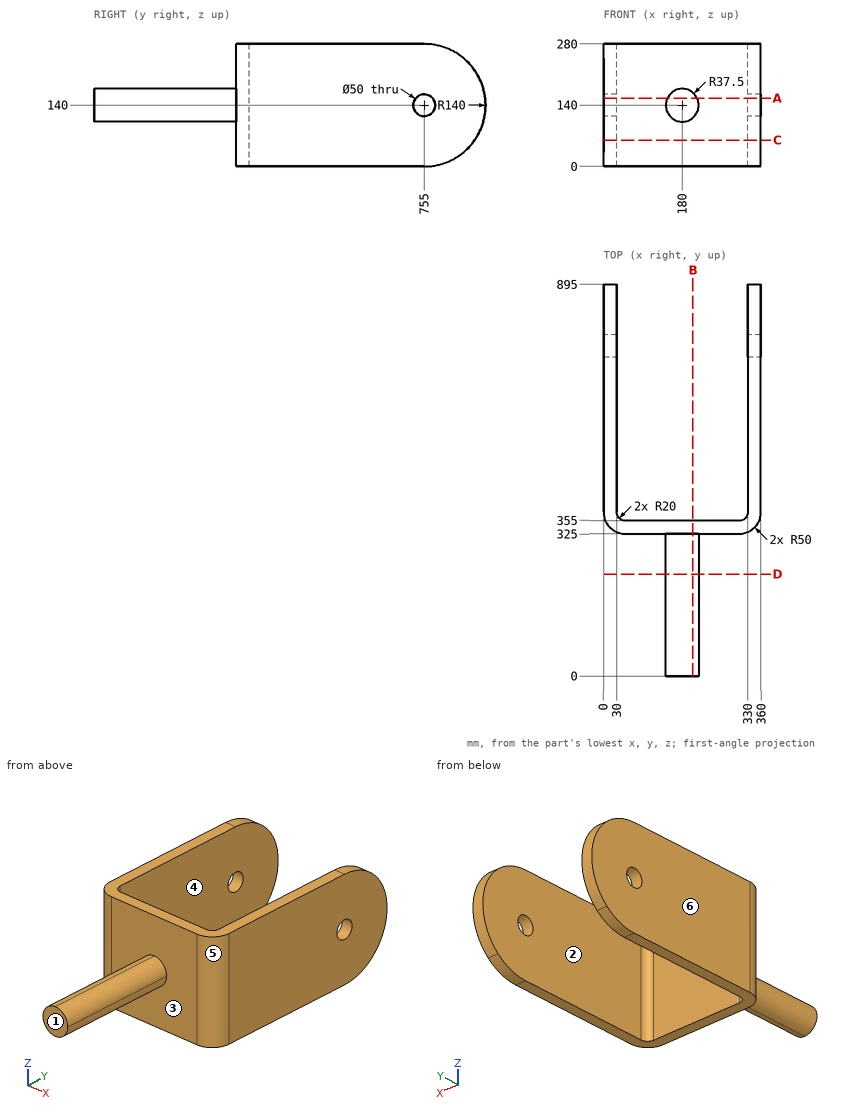
Can you work these out from the drawing? Everything is in mm from the part's minimum corner. A direction names the side the tool comes from. Round coordinates to 2 decimals unless told otherwise and drop trailing zeros. Loops run counter-clockwise (first coordinate to the right, second up) from the corner with the lowest first, then second, coordinate; pieces in that order, holes last. Notation, with made-up numbers: (1.25, -22.75) - (27.25, -22.75) arc R10 cw to (27.25, -18.75) - close; hole circle Ø2 at (18, 40.5). An arc over 180 degrees is marked (long way). Answer in a Markdown table with one row per item. Add a question column.
(1) If we section it at C-C (z = 60): Please give me the cut outline in (x, y), plus the area to 3 significant figures.
(2) If we mould it in two halves opening along X, with no side actions, what happens to the marked faces 4, 5 and 6? For each: pulls with the +X half, pulls with the -X half, needs draft (parallel to the pull), parting line crosses it, or undercut.
(3) I need wall thicknesses on line 1 along X through (y, z) = (641, 182.5); line 2 along Z through (x, y) = (17, 755); line 3 along Y through (x, z) = (135.5, 106.5). Which ranges of each line are inside material? Lowest first, please.
(4) If we section it at A-A (z = 156): Please give me the cut outline in (x, y).
(5) For the marked faces 1, 2 and 3, which set-ups out of +Z, -Z, +X, -X, +Y, -Y let a thin tool reach every point of the face, with its end or its side?
(6) I'm going to push flat-ended pins straight in: pin 1 (1 mm diameter, centred on x = 129.5, z = 216, fed in from -Y); pin 2 (3 mm diameter, centred on x = 209, z = 94, fed in from +Y); pin 3 (6 mm diameter, centred on y = 125.5, z = 131, fed in from -X). Where does each tip first touch, or does it pass through?
(7) If we section it at B-B (x = 204.5): Please give me the cut outline in (y, z).
(8) If we section it at D-D (y = 233): Please give me the cut outline in (x, z).
Model answer:
| question | item | result |
|---|---|---|
| 1 | outline | (0, 375) arc R50 ccw to (50, 325) - (310, 325) arc R50 ccw to (360, 375) - (360, 869.89) - (330, 869.89) - (330, 375) arc R20 cw to (310, 355) - (50, 355) arc R20 cw to (30, 375) - (30, 869.89) - (0, 869.89) - close |
| 1 | area | 40,800 mm² |
| 2 | face 4 | undercut |
| 2 | face 5 | pulls with the +X half |
| 2 | face 6 | pulls with the -X half |
| 3 | line 1 | x = 0 to 30, 330 to 360 |
| 3 | line 2 | z = 0 to 115, 165 to 280 |
| 3 | line 3 | y = 325 to 355 |
| 4 | outline | (0, 375) arc R50 ccw to (50, 325) - (146.08, 325) - (146.08, 0) - (213.92, 0) - (213.92, 325) - (310, 325) arc R50 ccw to (360, 375) - (360, 735.79) - (330, 735.79) - (330, 375) arc R20 cw to (310, 355) - (50, 355) arc R20 cw to (30, 375) - (30, 735.79) - (0, 735.79) - close; (0, 774.21) - (30, 774.21) - (30, 894.08) - (0, 894.08) - close; (330, 774.21) - (360, 774.21) - (360, 894.08) - (330, 894.08) - close |
| 5 | face 1 | +Z, -Z, +X, -X, -Y |
| 5 | face 2 | +Z, -Z, +Y |
| 5 | face 3 | -Y |
| 6 | pin 1 | stops at y = 325 |
| 6 | pin 2 | stops at y = 355 |
| 6 | pin 3 | stops at x = 142.98 |
| 7 | outline | (0, 111.61) - (325, 111.61) - (325, 0) - (355, 0) - (355, 280) - (325, 280) - (325, 168.39) - (0, 168.39) - close |
| 8 | outline | circle Ø75 at (180, 140) |
